The listing builds one solid part. Answer for the finished solid, in the listing's coordinates (mm). A direction names the side the tool comes from. Coordinates: 2 decimals unless noted, no trailing zeros. Loops run counter-clockwise (first coordinate to the right, second up) from the corner with the lowest first, then second, coordinate; pieces in that order, holes last. Notation, with made-up numbers: (-9, 39) - (50, 39) arc R21 cw to (50, 75) - close; hole circle Ø2 at (45.5, 49). An arc over 180 degrees is marked (long way). One line per question, with ' | ' between items.
from build123d import *

# Parameters (mm, degrees)
BASE_PLATE_SKETCH_W         = 150
BASE_PLATE_SKETCH_H         = 120
BASE_PLATE_150X120X15_DEPTH = 15
RAISED_BOSS_SKETCH_R        = 12.5
RAISED_BOSS_SKETCH_R_2      = 7.5
RAISED_BOSS_15MM_DEPTH      = 15
BEARING_BLOCK_DEPTH         = 20
RELIEF_CUT_SKETCH_W         = 25
RELIEF_CUT_SKETCH_H         = 30
RELIEF_CUT_DEPTH            = 15
PLATE_CORNER_FILLETS_R25_R  = 25
BLOCK_SLOT_SKETCH_W         = 30
BLOCK_SLOT_SKETCH_H         = 10
BLOCK_SLOT_30X10_DEPTH      = 15
SUPPORT_RIB_DEPTH           = 6
BEARING_BORE_SKETCH_R       = 12.5
BEARING_BORE_25_DEPTH       = 15


with BuildPart() as part:
    # Base Plate Sketch → Base Plate 150x120x15 (new body)
    with BuildSketch(Plane.XY):
        with Locations((75, 60)):
            Rectangle(BASE_PLATE_SKETCH_W, BASE_PLATE_SKETCH_H)
    extrude(amount=BASE_PLATE_150X120X15_DEPTH)

    # Raised Boss Sketch → Raised Boss 15mm (add)
    # profile 1 of 4: a face of its own
    with BuildSketch(Plane.XY.offset(15)):
        with Locations((25, 95)):
            Circle(RAISED_BOSS_SKETCH_R)
        with Locations((25, 95)):
            Circle(RAISED_BOSS_SKETCH_R_2, mode=Mode.SUBTRACT)
    # profile 2 of 4: a face of its own
    with BuildSketch(Plane.XY.offset(15)):
        with Locations((125, 95)):
            Circle(RAISED_BOSS_SKETCH_R)
        with Locations((125, 95)):
            Circle(RAISED_BOSS_SKETCH_R_2, mode=Mode.SUBTRACT)
    # profile 3 of 4: a face of its own
    with BuildSketch(Plane.XY.offset(15)):
        with Locations((125, 25)):
            Circle(RAISED_BOSS_SKETCH_R)
        with Locations((125, 25)):
            Circle(RAISED_BOSS_SKETCH_R_2, mode=Mode.SUBTRACT)
    # profile 4 of 4: a face of its own
    with BuildSketch(Plane.XY.offset(15)):
        with Locations((25, 25)):
            Circle(RAISED_BOSS_SKETCH_R)
        with Locations((25, 25)):
            Circle(RAISED_BOSS_SKETCH_R_2, mode=Mode.SUBTRACT)
    extrude(amount=RAISED_BOSS_15MM_DEPTH)

    # Bearing Block Sketch → Bearing Block (add, symmetric)
    with BuildSketch(Plane(origin=(0, 60, 0), x_dir=(1, 0, 0), z_dir=(0, 1, 0))):
        with BuildLine():
            Line((50, -40), (50, -15))
            Line((50, -15), (100, -15))
            Line((100, -15), (100, -40))
            ThreePointArc((100, -40), (75, -65), (50, -40))
        make_face()
    extrude(amount=BEARING_BLOCK_DEPTH, both=True)

    # Relief Cut Sketch → Relief Cut (cut)
    with BuildSketch(Plane.XY.offset(15)):
        Polygon((150, 60), (150, 75), (125, 75), (125, 45), (150, 45), align=None)
        with Locations((12.5, 60)):
            Rectangle(RELIEF_CUT_SKETCH_W, RELIEF_CUT_SKETCH_H)
    extrude(amount=-RELIEF_CUT_DEPTH, mode=Mode.SUBTRACT)

    # Plate Corner Fillets R25
    plate_corner_fillets_r25_edges = [part.edges().sort_by_distance(p)[0] for p in [
        (0, 120, 7.5),
        (150, 120, 7.5),
        (150, 0, 7.5),
        (0, 0, 7.5),
    ]]
    fillet(plate_corner_fillets_r25_edges, radius=PLATE_CORNER_FILLETS_R25_R)

    # Block Slot Sketch → Block Slot 30x10 (cut)
    with BuildSketch(Plane.XY.offset(65)):
        with Locations((75, 60)):
            Rectangle(BLOCK_SLOT_SKETCH_W, BLOCK_SLOT_SKETCH_H)
    extrude(amount=-BLOCK_SLOT_30X10_DEPTH, mode=Mode.SUBTRACT)

    # Support Rib Sketch → Support Rib (add, symmetric)
    with BuildSketch(Plane(origin=(75, 0, 0), x_dir=(0, 0, -1), z_dir=(1, 0, 0))):
        Polygon((-15, 0), (-65, 40), (-15, 40), align=None)
    extrude(amount=SUPPORT_RIB_DEPTH, both=True)

    # Bearing Bore Sketch → Bearing Bore Ø25 (cut)
    with BuildSketch(Plane(origin=(0, 80, 0), x_dir=(1, 0, 0), z_dir=(0, 1, 0))):
        with Locations(Location((75, -40, 0), (0, 0, 270))):
            Circle(BEARING_BORE_SKETCH_R)
    extrude(amount=-BEARING_BORE_25_DEPTH, mode=Mode.SUBTRACT)


solid = part.part
Item 1: Which of the six approach directions +Z, -Z, +X, -X, +Y, -Y give full straight-line access (tool end or side, diameter ignored) to faces 4 (the face through (90, 60, 55)), 5 (the face through (25, 17, 30)), 6 (the face through (25, 60, 8))?
Taken from the geometry:
face 4: +Z | face 5: +Z, -X, +Y, -Y | face 6: +Z, -Z, -X
Item 2: Find section D-D, the plane y = 52.5. Write down the section's boundary in (x, z).
Taken from the geometry:
outline: (25, 0) - (125, 0) - (125, 15) - (100, 15) - (100, 40) arc R25 ccw to (50, 40) - (50, 15) - (25, 15) - close
Item 3: Find section C-C, the plane z = 10.5. Write down the section's boundary in (x, y), plus the area to 3 significant figures.
Taken from the geometry:
outline: (0, 25) arc R25 ccw to (25, 0) - (125, 0) arc R25 ccw to (150, 25) - (150, 45) - (125, 45) - (125, 75) - (150, 75) - (150, 95) arc R25 ccw to (125, 120) - (25, 120) arc R25 ccw to (0, 95) - (0, 75) - (25, 75) - (25, 45) - (0, 45) - close | area: 16,000 mm2
Item 4: Find the intervals of material crossed by line 1 (Y direction, x = 25, z = 25.25); line 2 (Z direction, x = 75, y = 71.25); line 3 (Z direction, x = 37, y = 79), in increasing order. Write a range as [from, to].
Taken from the geometry:
line 1: y = [12.5, 17.5], [32.5, 37.5], [82.5, 87.5], [102.5, 107.5] | line 2: z = [0, 27.5], [52.5, 65] | line 3: z = [0, 15]
Item 5: Find section A-A, the plane y = 73. Write down the section's boundary in (x, z).
Taken from the geometry:
outline: (25, 0) - (125, 0) - (125, 15) - (100, 15) - (100, 40) arc R25 ccw to (50, 40) - (50, 15) - (25, 15) - close; hole circle Ø25 at (75, 40)
Item 6: The mould has two halves that part along Y. Classify faces 1 (the face through (100, 60, 27)), 2 (the face through (80.9, 80, 28.5)), 3 (the face through (23.37, 87.68, 22.4)): pulls with the +Y half, pulls with the -Y half, needs draft (parallel to the pull), parting line crosses it, or undercut.
Taken from the geometry:
face 1: needs draft | face 2: pulls with the +Y half | face 3: undercut
Item 7: Each of these flat-tipped pins is pushed along its axis until it touches: pin 1 Ø4.5 at (x, y) = (24.5, 22.5) entering from +Z; pin 2 Ø8 at (y, z) = (73, 34) entering from +X; pin 3 Ø12.5 at (x, y) = (126, 93) entering from +Z; pin 4 Ø1.5 at (x, y) = (111.5, 30) entering from -Z. Where does it stop, or does it pass through?
Taken from the geometry:
pin 1: stops at z = 15 | pin 2: stops at x = 100 | pin 3: stops at z = 30 | pin 4: stops at z = 0
Item 8: Find section B-B, the plane x = 130.5. Write down the section's boundary in (y, z), plus the area to 3 significant figures.
Taken from the geometry:
outline: (0.61, 0) - (45, 0) - (45, 15) - (36.22, 15) - (36.22, 30) - (30.1, 30) - (30.1, 15) - (19.9, 15) - (19.9, 30) - (13.78, 30) - (13.78, 15) - (0.61, 15) - close; (75, 0) - (119.39, 0) - (119.39, 15) - (106.22, 15) - (106.22, 30) - (100.1, 30) - (100.1, 15) - (89.9, 15) - (89.9, 30) - (83.78, 30) - (83.78, 15) - (75, 15) - close | area: 1,700 mm2
